```python
from build123d import *

# Parameters (mm, degrees)
SKETCH_1_R          = 10
EXTRUDE_1_DEPTH     = 10
SKETCH_2_W          = 29.5
SKETCH_2_H          = 29.5
EXTRUDE_2_DEPTH     = 5
SKETCH_3_R          = 10.5
EXTRUDE_3_DEPTH     = 17
SKETCH_4_R          = 2.25
CUT_EXTRUDE_1_DEPTH = 17
FILLET_1_R          = 1


with BuildPart() as part:
    # 草图1 → 凸台-拉伸1 (new body)
    with BuildSketch(Plane(origin=(0, 0, 0), x_dir=(1, 0, 0), z_dir=(0, 1, 0))):
        with Locations(Location((0, 0, 0), (0, 0, 270))):
            Circle(SKETCH_1_R)
    extrude(amount=EXTRUDE_1_DEPTH)

    # 草图2 → 凸台-拉伸2 (add)
    with BuildSketch(Plane(origin=(0, 10, 0), x_dir=(1, 0, 0), z_dir=(0, 1, 0))):
        Rectangle(SKETCH_2_W, SKETCH_2_H)
    extrude(amount=EXTRUDE_2_DEPTH)

    # 草图3 → 凸台-拉伸3 (add)
    with BuildSketch(Plane(origin=(0, 15, 0), x_dir=(1, 0, 0), z_dir=(0, 1, 0))):
        with Locations(Location((0, 0, 0), (0, 0, 270))):
            Circle(SKETCH_3_R)
    extrude(amount=EXTRUDE_3_DEPTH)

    # 草图4 → 切除-拉伸1 (cut)
    with BuildSketch(Plane(origin=(0, 15, 0), x_dir=(1, 0, 0), z_dir=(0, 1, 0))):
        with Locations(Location((11, 11, 0), (0, 0, 270))):
            Circle(SKETCH_4_R)
        with Locations(Location((-11, 11, 0), (0, 0, 270))):
            Circle(SKETCH_4_R)
        with Locations(Location((-11, -11, 0), (0, 0, 270))):
            Circle(SKETCH_4_R)
        with Locations(Location((11, -11, 0), (0, 0, 270))):
            Circle(SKETCH_4_R)
    extrude(amount=-CUT_EXTRUDE_1_DEPTH, mode=Mode.SUBTRACT)

    # 圆角1
    fillet_1_edges = [part.edges().sort_by_distance(p)[0] for p in [
        (14.75, 12.5, 14.75),
        (14.75, 12.5, -14.75),
        (-14.75, 12.5, -14.75),
        (-14.75, 12.5, 14.75),
    ]]
    fillet(fillet_1_edges, radius=FILLET_1_R)


solid = part.part
```
Can you work these out from the model? Positions are in its coordinate system, mm. A direction names the side the tool comes from. Give positions to 0.01 mm unless a question says otherwise; leave off trailing zeros. Order: outer loops, then holes, each group sorted by start corner. A loop starts at its lowest first (then second) coordinate and runs counter-clockwise, first axis right, second up. Notation, with made-up numbers: (-24, 13) - (3, 13) arc R28 cw to (3, 48) - close; hole circle Ø3 at (-6, 49). An arc over 180 degrees is marked (long way). Use a Markdown table: item, result. Add a question column.
Q1. If we mould it in two halves opening along Z, with no side actions, what happens to faces 3 (the cylindrical face through (-9.76, 4.93, -2.17)), 4 (the cylindrical face through (-14.465, 12.535, 14.449)), 5 (the cylindrical face through (12.52, 12.54, 9.34)), 6 (the flat face through (-3, 10, -10))? For each: released by +Z, released by -Z, zero draft, split by the parting line, or undercut.
Q2. If we section it at A-A on x = 11: Write out the boundary of the cut face in (y, z).
Q3. If we section it at B-B on z = -11: Write out the boundary of the cut face in (x, y), plus the area to 4 significant figures.
Q4. If we section it at D-D on z = 0: Write out the boundary of the cut face in (x, y).
Q5. I'm going to push flat-ended pins straight in: pin 1 (3 mm diameter, centred on y = 5, z = 6, fed in from +X); pin 2 (3.5 mm diameter, centred on x = 11, z = 11, fed in from +Y); pin 3 (6 mm diameter, centred on x = -11, z = -11, fed in from +Y); pin 4 (4 mm diameter, centred on y = 18.5, z = -11, fed in from +X). Where does each tip first touch, or does it pass through?
Q6. Please list where these lines run through material, in increasing order: line 1 along X through (y, z) = (12.9, 11); line 2 along Y through (x, z) = (12, 8.25); line 3 along Z through (x, y) = (-0.5, 21.5).
Q7. If we section it at C-C on x = 0: Write out the boundary of the cut face in (y, z).
Q8. On a 3-axis mill with a long thin cutter (end or side, diameter ignored), from which of +Z, -Z, +X, -X, +Y, -Y can I reach the whole of each face in a straight line? I mean faces 1 (the cylindrical face through (14.449, 12.535, -14.465)), 2 (the cylindrical face through (3.2, 23.4, 10)). Say none if no direction works.
Answers follow:
| question | item | result |
|---|---|---|
| 1 | face 3 | split by the parting line |
| 1 | face 4 | released by +Z |
| 1 | face 5 | undercut |
| 1 | face 6 | zero draft |
| 2 | outline | (10, -14.75) - (15, -14.75) - (15, -13.25) - (10, -13.25) - close; (10, -8.75) - (15, -8.75) - (15, 8.75) - (10, 8.75) - close; (10, 13.25) - (15, 13.25) - (15, 14.75) - (10, 14.75) - close |
| 3 | outline | (-14.75, 10) - (-13.25, 10) - (-13.25, 15) - (-14.75, 15) - close; (-8.75, 10) - (8.75, 10) - (8.75, 15) - (-8.75, 15) - close; (13.25, 10) - (14.75, 10) - (14.75, 15) - (13.25, 15) - close |
| 3 | area | 102.5 mm^2 |
| 4 | outline | (-14.75, 10) - (-10, 10) - (-10, 0) - (10, 0) - (10, 10) - (14.75, 10) - (14.75, 15) - (10.5, 15) - (10.5, 32) - (-10.5, 32) - (-10.5, 15) - (-14.75, 15) - close |
| 5 | pin 1 | stops at x = 8.93 |
| 5 | pin 2 | passes through |
| 5 | pin 3 | stops at y = 15 |
| 5 | pin 4 | stops at x = 5.41 |
| 6 | line 1 | x = -14.75 to -13.25, -8.75 to 8.75, 13.25 to 14.75 |
| 6 | line 2 | y = 10 to 15 |
| 6 | line 3 | z = -10.49 to 10.49 |
| 7 | outline | (0, -10) - (10, -10) - (10, -14.75) - (15, -14.75) - (15, -10.5) - (32, -10.5) - (32, 10.5) - (15, 10.5) - (15, 14.75) - (10, 14.75) - (10, 10) - (0, 10) - close |
| 8 | face 1 | -Z, +X, +Y, -Y |
| 8 | face 2 | +Y |
